Verification items for the finished model (mm, model axes). Face numbers are marked on the shaded views. A direction names the side the tool comes from. Coordinates: 2 decimals unless noted, no trailing zeros. Write each loop counter-clockwise with the first axis right and the second up, starting at its lowest first coordinate (ties: lowest second). Pieces come first, ordered by that corner, then holes.
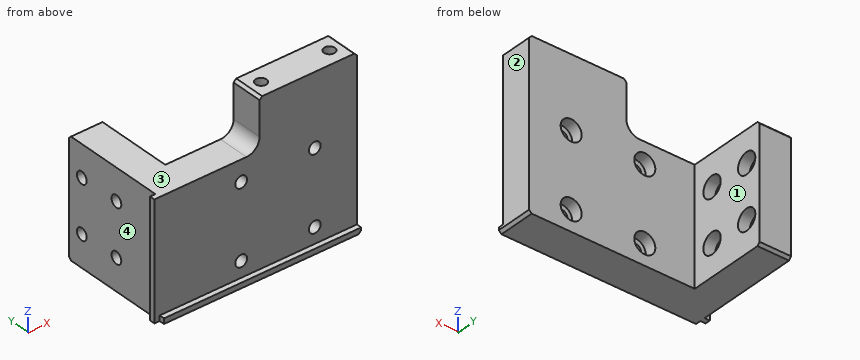
```python
from build123d import *

# Parameters (mm, degrees)
SKETCH1_W                                           = 75
SKETCH1_H                                           = 12
BOSS_EXTRUDE1_DEPTH                                 = 73
SKETCH2_W                                           = 75
SKETCH2_H                                           = 2
BOSS_EXTRUDE2_DEPTH                                 = 2
SKETCH3_W                                           = 75
SKETCH3_H                                           = 10
BOSS_EXTRUDE3_DEPTH                                 = 15
SKETCH4_W                                           = 12
SKETCH4_H                                           = 63
BOSS_EXTRUDE4_DEPTH                                 = 30
SKETCH5_W                                           = 63
SKETCH5_H                                           = 2
BOSS_EXTRUDE5_DEPTH                                 = 2
SKETCH7_W                                           = 40
SKETCH7_H                                           = 42
CUT_EXTRUDE2_DEPTH                                  = 29
M5_TAPPED_HOLE1_D                                   = 4.2
M5_TAPPED_HOLE1_DEPTH                               = 12.4
M5_TAPPED_HOLE1_TIP                                 = 1.2618073
CBORE_FOR_M4_HEX_SOCKET_HEAD_CAP_SCREW1_D           = 4.5
CBORE_FOR_M4_HEX_SOCKET_HEAD_CAP_SCREW1_CBORE_D     = 8
CBORE_FOR_M4_HEX_SOCKET_HEAD_CAP_SCREW1_CBORE_DEPTH = 4.4
SKETCH12_W                                          = 37
SKETCH12_H                                          = 10
CUT_EXTRUDE3_DEPTH                                  = 88.92184029
M5_TAPPED_HOLE2_D                                   = 4.2
M5_TAPPED_HOLE2_DEPTH                               = 12.4
M5_TAPPED_HOLE2_TIP                                 = 1.2618073
FILLET1_R                                           = 5
CBORE_FOR_M4_HEX_SOCKET_HEAD_CAP_SCREW2_D           = 4.5
CBORE_FOR_M4_HEX_SOCKET_HEAD_CAP_SCREW2_CBORE_D     = 8
CBORE_FOR_M4_HEX_SOCKET_HEAD_CAP_SCREW2_CBORE_DEPTH = 4.4
CHAMFER1_SIZE                                       = 1


with BuildPart() as part:
    # Sketch1 → Boss-Extrude1 (new body)
    with BuildSketch(Plane.XY):
        Rectangle(SKETCH1_W, SKETCH1_H)
    extrude(amount=BOSS_EXTRUDE1_DEPTH)

    # Sketch2 → Boss-Extrude2 (add)
    with BuildSketch(Plane.XZ.offset(6)):
        with Locations((0, 1)):
            Rectangle(SKETCH2_W, SKETCH2_H)
    extrude(amount=BOSS_EXTRUDE2_DEPTH)

    # Sketch3 → Boss-Extrude3 (add)
    with BuildSketch(Plane(origin=(0, 6, 0), x_dir=(1, 0, 0), z_dir=(0, 1, 0))):
        with Locations((0, -68)):
            Rectangle(SKETCH3_W, SKETCH3_H)
    extrude(amount=BOSS_EXTRUDE3_DEPTH)

    # Sketch4 → Boss-Extrude4 (add)
    with BuildSketch(Plane(origin=(0, 6, 0), x_dir=(1, 0, 0), z_dir=(0, 1, 0))):
        with Locations((-31.5, -31.5)):
            Rectangle(SKETCH4_W, SKETCH4_H)
    extrude(amount=BOSS_EXTRUDE4_DEPTH)

    # Sketch5 → Boss-Extrude5 (add)
    with BuildSketch(Plane.ZY.offset(37.5)):
        with Locations((31.5, -5)):
            Rectangle(SKETCH5_W, SKETCH5_H)
    extrude(amount=BOSS_EXTRUDE5_DEPTH)

    # Sketch7 → Cut-Extrude2 (cut)
    with BuildSketch(Plane.XY.offset(73)):
        with Locations((-19.5, 15)):
            Rectangle(SKETCH7_W, SKETCH7_H)
    extrude(amount=-CUT_EXTRUDE2_DEPTH, mode=Mode.SUBTRACT)

    # M5 Tapped Hole1
    with Locations(Plane.XY.offset(73)):
        with Locations((19, 10)):
            Hole(M5_TAPPED_HOLE1_D / 2, depth=M5_TAPPED_HOLE1_DEPTH)
            with Locations((0, 0, -(M5_TAPPED_HOLE1_DEPTH + M5_TAPPED_HOLE1_TIP / 2))):  # 118° drill point
                Cone(0, M5_TAPPED_HOLE1_D / 2, M5_TAPPED_HOLE1_TIP, mode=Mode.SUBTRACT)

    # CBORE for M4 Hex Socket Head Cap Screw1 (through all)
    with Locations(Plane(origin=(-25.5, 0, 0), x_dir=(0, 0, -1), z_dir=(1, 0, 0))):
        with Locations((-32, 30), (-32, 14), (-12, 14), (-12, 30)):
            CounterBoreHole(CBORE_FOR_M4_HEX_SOCKET_HEAD_CAP_SCREW1_D / 2, CBORE_FOR_M4_HEX_SOCKET_HEAD_CAP_SCREW1_CBORE_D / 2, CBORE_FOR_M4_HEX_SOCKET_HEAD_CAP_SCREW1_CBORE_DEPTH)

    # Sketch12 → Cut-Extrude3 (cut, through all)
    with BuildSketch(Plane(origin=(0, 21, 0), x_dir=(1, 0, 0), z_dir=(0, 1, 0))):
        with Locations((19, -68)):
            Rectangle(SKETCH12_W, SKETCH12_H)
    extrude(amount=-CUT_EXTRUDE3_DEPTH, mode=Mode.SUBTRACT)

    # M5 Tapped Hole2
    with Locations(Plane.XY.offset(63)):
        with Locations((32, 0), (6, 0)):
            Hole(M5_TAPPED_HOLE2_D / 2, depth=M5_TAPPED_HOLE2_DEPTH)
            with Locations((0, 0, -(M5_TAPPED_HOLE2_DEPTH + M5_TAPPED_HOLE2_TIP / 2))):  # 118° drill point
                Cone(0, M5_TAPPED_HOLE2_D / 2, M5_TAPPED_HOLE2_TIP, mode=Mode.SUBTRACT)

    # Fillet1
    fillet1_edges = [part.edges().sort_by_distance(p)[0] for p in [
        (0.5, 0, 44),
    ]]
    fillet(fillet1_edges, radius=FILLET1_R)

    # CBORE for M4 Hex Socket Head Cap Screw2 (through all)
    with Locations(Plane(origin=(0, 6, 0), x_dir=(1, 0, 0), z_dir=(0, 1, 0))):
        with Locations((-6.5, -8), (21.5, -8), (-6.5, -36), (21.5, -36)):
            CounterBoreHole(CBORE_FOR_M4_HEX_SOCKET_HEAD_CAP_SCREW2_D / 2, CBORE_FOR_M4_HEX_SOCKET_HEAD_CAP_SCREW2_CBORE_D / 2, CBORE_FOR_M4_HEX_SOCKET_HEAD_CAP_SCREW2_CBORE_DEPTH)

    # Chamfer1
    chamfer1_edges = [part.edges().sort_by_distance(p)[0] for p in [
        (0.5, 0, 63),
        (37.5, 0, 63),
        (37.5, -1, 0),
        (-31.5, 36, 0),
        (-31.5, 36, 44),
    ]]
    chamfer(chamfer1_edges, length=CHAMFER1_SIZE)


solid = part.part
```
1. Sectioned sample at C-C, the plane x = -29. Record the boundary of the cut face in (y, z), and give its area (3 significant figures).
2. Sectioned sample at A-A, the plane y = 30. Record the boundary of the cut face in (x, z), and give its area (3 significant figures).
3. Tool access check on the marked faces 1, 2, 3 and 4. Record the directions out of +Z, -Z, +X, -X, +Y, -Y that give a thin tool (end or side, any length) a straight path to the whole face; none if there is none.
4. Sectioned sample at B-B, the plane x = 21.5. Record the boundary of the cut face in (y, z), and give its area (3 significant figures).
5. Material ranges on L1, parallel to Y at x = -28, z = 32; L2, parallel to X at y = 3.7, z = 36; L3, parallel to Y at x = -29.5, z = 31, recorded low to high.
6. Sectioned sample at D-D, the plane z = 23. Record the boundary of the cut face in (x, y), and give its area (3 significant figures).
7. Gauge pin test, flat ends, axial feed: P1, Ø6.5, axis at y = 14, z = 32, coming from the -X side; P2, Ø13, axis at x = -6.5, z = 8, coming from the +Y side; P3, Ø2.5, axis at x = 23, z = 8, coming from the +Y side. Record the tip position at first contact, or that the pin passes through.
Outcome:
1. outline: (-8, 0) - (35, 0) - (36, 1) - (36, 43) - (35, 44) - (-6, 44) - (-6, 2) - (-8, 2) - close; hole circle Ø8 at (14, 12); hole circle Ø8 at (14, 32); hole circle Ø8 at (30, 12); hole circle Ø8 at (30, 32)
1. area: 1,650 mm2
2. outline: (-37.5, 0) - (-25.5, 0) - (-25.5, 8) - (-29.9, 8) - (-29.9, 9.75) - (-37.5, 9.75) - close; (-37.5, 14.25) - (-29.9, 14.25) - (-29.9, 16) - (-25.5, 16) - (-25.5, 28) - (-29.9, 28) - (-29.9, 29.75) - (-37.5, 29.75) - close; (-37.5, 34.25) - (-29.9, 34.25) - (-29.9, 36) - (-25.5, 36) - (-25.5, 44) - (-37.5, 44) - close
2. area: 389 mm2
3. face 1: +Z, -Z, +X, +Y
3. face 2: +Z, -Z, +X, +Y, -Y
3. face 3: +Z, -X, +Y, -Y
3. face 4: +Z, -Z, -X, +Y
4. outline: (-8, 0) - (6, 0) - (6, 4) - (1.6, 4) - (1.6, 5.75) - (-6, 5.75) - (-6, 2) - (-8, 2) - close; (-6, 10.25) - (1.6, 10.25) - (1.6, 12) - (6, 12) - (6, 32) - (1.6, 32) - (1.6, 33.75) - (-6, 33.75) - close; (-6, 38.25) - (1.6, 38.25) - (1.6, 40) - (6, 40) - (6, 63) - (-6, 63) - close
4. area: 621 mm2
5. L1: y = -6 to 10, 18 to 26, 34 to 36
5. L2: x = -37.5 to -10.5, -2.5 to 17.5, 25.5 to 37.5
5. L3: y = -6 to 10.13, 17.87 to 26.13, 33.87 to 36
6. outline: (-39.5, -6) - (37.5, -6) - (37.5, 6) - (-25.5, 6) - (-25.5, 36) - (-37.5, 36) - (-37.5, -4) - (-39.5, -4) - close
6. area: 1,260 mm2
7. P1: stops at x = -37.5
7. P2: stops at y = 6
7. P3: stops at y = 1.6
